Part model, mm, in its own coordinate system. A direction names the side the tool comes from. Give positions to 0.01 mm unless a question says otherwise; leave off trailing zeros. Loops run counter-clockwise (first coordinate to the right, second up) from the corner with the lowest first, then second, coordinate; pieces in that order, holes last. Notation, with made-up numbers: M 5,77 L 36,77 A36 cw 36,114 Z; hole C -6.75,-33.5 d1. An arc over 180 degrees is marked long. Answer in a Markdown table with one row per item.
from build123d import *

# Parameters (mm, degrees)
SKETCH_1_W             = 100
SKETCH_1_H             = 95
EXTRUDE_1_DEPTH        = 25
SKETCH_2_R             = 31
CUT_EXTRUDE_1_DEPTH    = 22
SKETCH_3_R             = 27
CUT_EXTRUDE_2_DEPTH    = 73.389571072
CUT_EXTRUDE_START      = 16
SKETCH_4_R             = 32.5
CUT_EXTRUDE_3_DEPTH    = 2.1
HOLE_WIZARD_M8_1_D     = 6.8
HOLE_WIZARD_M8_1_DEPTH = 15.75
HOLE_WIZARD_M8_1_TIP   = 2.042926105
HOLE_WIZARD_M8_2_D     = 6.8
HOLE_WIZARD_M8_2_DEPTH = 15.75
HOLE_WIZARD_M8_2_TIP   = 2.042926105
CHAMFER_1_SIZE         = 10
CHAMFER_2_SIZE         = 1
HOLE_WIZARD_M8_3_D     = 6.8
HOLE_WIZARD_M8_3_DEPTH = 19.75
HOLE_WIZARD_M8_3_TIP   = 2.042926105


with BuildPart() as part:
    # 草图1 → 凸台-拉伸1 (new body)
    with BuildSketch(Plane(origin=(0, 0, 0), x_dir=(0, 0, -1), z_dir=(1, 0, 0))):
        Rectangle(SKETCH_1_W, SKETCH_1_H)
    extrude(amount=EXTRUDE_1_DEPTH)

    # 草图2 → 切除-拉伸1 (cut)
    with BuildSketch(Plane.ZY):
        with Locations((0, 7.5)):
            Circle(SKETCH_2_R)
    extrude(amount=-CUT_EXTRUDE_1_DEPTH, mode=Mode.SUBTRACT)

    # 草图3 → 切除-拉伸2 (cut, through all)
    with BuildSketch(Plane.ZY.offset(-22)):
        with Locations((0, 7.5)):
            Circle(SKETCH_3_R)
    extrude(amount=-CUT_EXTRUDE_2_DEPTH, mode=Mode.SUBTRACT)

    # 草图4 → 切除-拉伸3 (cut)
    with BuildSketch(Plane.ZY.offset(-22).offset(CUT_EXTRUDE_START)):
        with Locations((0, 7.5)):
            Circle(SKETCH_4_R)
    extrude(amount=CUT_EXTRUDE_3_DEPTH, mode=Mode.SUBTRACT)

    # M8 螺纹孔1
    with Locations(Plane.XY.offset(50)):
        with Locations((12.5, 17.5)):
            Hole(HOLE_WIZARD_M8_1_D / 2, depth=HOLE_WIZARD_M8_1_DEPTH)
            with Locations((0, 0, -(HOLE_WIZARD_M8_1_DEPTH + HOLE_WIZARD_M8_1_TIP / 2))):  # 118° drill point
                Cone(0, HOLE_WIZARD_M8_1_D / 2, HOLE_WIZARD_M8_1_TIP, mode=Mode.SUBTRACT)

    # M8 螺纹孔2
    with Locations(Plane(origin=(0, 0, -50), x_dir=(-1, 0, 0), z_dir=(0, 0, -1))):
        with Locations((-12.5, 17.5)):
            Hole(HOLE_WIZARD_M8_2_D / 2, depth=HOLE_WIZARD_M8_2_DEPTH)
            with Locations((0, 0, -(HOLE_WIZARD_M8_2_DEPTH + HOLE_WIZARD_M8_2_TIP / 2))):  # 118° drill point
                Cone(0, HOLE_WIZARD_M8_2_D / 2, HOLE_WIZARD_M8_2_TIP, mode=Mode.SUBTRACT)

    # 倒角1
    chamfer_1_edges = [part.edges().sort_by_distance(p)[0] for p in [
        (12.5, 47.5, 50),
        (12.5, 47.5, -50),
    ]]
    chamfer(chamfer_1_edges, length=CHAMFER_1_SIZE)

    # 倒角2
    chamfer_2_edges = [part.edges().sort_by_distance(p)[0] for p in [
        (12.5, -47.5, -50),
        (12.5, -47.5, 50),
    ]]
    chamfer(chamfer_2_edges, length=CHAMFER_2_SIZE)

    # M8 螺纹孔3
    with Locations(Plane(origin=(0, -47.5, 0), x_dir=(-1, 0, 0), z_dir=(0, -1, 0))):
        with Locations((-12.5, -40), (-12.5, 0), (-12.5, 40)):
            Hole(HOLE_WIZARD_M8_3_D / 2, depth=HOLE_WIZARD_M8_3_DEPTH)
            with Locations((0, 0, -(HOLE_WIZARD_M8_3_DEPTH + HOLE_WIZARD_M8_3_TIP / 2))):  # 118° drill point
                Cone(0, HOLE_WIZARD_M8_3_D / 2, HOLE_WIZARD_M8_3_TIP, mode=Mode.SUBTRACT)


solid = part.part
(1) Drill centre lines: line 1 along Z through (x, y) = (12.5, -33.25); line 2 along Z through (x, y) = (13, -26.5); line 3 along X through (y, z) = (17.5, -43.75). Where is each one in solid material? Low to high.
Recorded:
| item | result |
|---|---|
| line 1 | z = -50 to -43.4, -36.6 to -3.4, 3.4 to 36.6, 43.4 to 50 |
| line 2 | z = -50 to -41.22, -38.78 to -1.22, 1.22 to 38.78, 41.22 to 50 |
| line 3 | x = 0 to 9.1, 15.9 to 25 |
(2) Pull direction Y, two halves, no side cores. Call faces 4 (the face through (12.06, -37.49, 36.63)), 5 (the face through (12.183, 17.998, -32.562)), 6 (the face through (11.955, -26.062, 0.226)): +Y half, -Y half, draft (parallel to the pull), parting line (faces both ways), or undercut.
Recorded:
| item | result |
|---|---|
| face 4 | draft |
| face 5 | undercut |
| face 6 | -Y half |
(3) Which spindle directions (+Z, -Z, +X, -X, +Y, -Y) get a long thin tool onto all of the face, cutting with end or side? Do faces 1 (the face through (1.923, -22.763, -6.72)), 2 (the face through (6, -4, 29)), 3 (the face through (13.24, 14.18, 42.01)). Say none if no direction does.
Recorded:
| item | result |
|---|---|
| face 1 | -X |
| face 2 | none |
| face 3 | +Z |
(4) Saw through at B-B (y = 7.5). Write the cut outline in (x, z), plus the area to 3 significant figures.
Recorded:
| item | result |
|---|---|
| outline | M 0,-50 L 25,-50 L 25,-27 L 22,-27 L 22,-31 L 6,-31 L 6,-32.5 L 3.9,-32.5 L 3.9,-31 L 0,-31 Z; M 0,31 L 3.9,31 L 3.9,32.5 L 6,32.5 L 6,31 L 22,31 L 22,27 L 25,27 L 25,50 L 0,50 Z |
| area | 968 mm^2 |
(5) Pin check, flat tips, straight feed: pin 1 Ø6 at (y, z) = (22.5, -15) entering from +X; pin 2 Ø6 at (x, z) = (12.5, -40) entering from -Y; pin 3 Ø6 at (x, y) = (12.5, 17.5) entering from -Z; pin 4 Ø4 at (y, z) = (1, -28) entering from -X. Stop position of each tip, or through.
Recorded:
| item | result |
|---|---|
| pin 1 | passes through |
| pin 2 | stops at y = -27.51 |
| pin 3 | stops at z = -34.01 |
| pin 4 | stops at x = 22 |
(6) Saw through at C-C (y = -31). Write the cut outline in (x, z).
Recorded:
| item | result |
|---|---|
| outline | M 0,-50 L 25,-50 L 25,50 L 0,50 Z; hole C 12.5,-40 d6.8; hole C 12.5,0 d6.8; hole C 12.5,40 d6.8 |
(7) Saw through at A-A (z = 15). Write the cut outline in (x, y), plus the area to 3 significant figures.
Recorded:
| item | result |
|---|---|
| outline | M 0,-47.5 L 25,-47.5 L 25,-14.95 L 22,-14.95 L 22,-19.63 L 6,-19.63 L 6,-21.33 L 3.9,-21.33 L 3.9,-19.63 L 0,-19.63 Z; M 0,34.63 L 3.9,34.63 L 3.9,36.33 L 6,36.33 L 6,34.63 L 22,34.63 L 22,29.95 L 25,29.95 L 25,47.5 L 0,47.5 Z |
| area | 1,040 mm^2 |
(8) Saw through at D-D (z = -29). Write the cut outline in (x, y), plus the area to 3 significant figures.
Recorded:
| item | result |
|---|---|
| outline | M 0,-47.5 L 25,-47.5 L 25,47.5 L 0,47.5 L 0,18.45 L 3.9,18.45 L 3.9,22.17 L 6,22.17 L 6,18.45 L 22,18.45 L 22,-3.45 L 6,-3.45 L 6,-7.17 L 3.9,-7.17 L 3.9,-3.45 L 0,-3.45 Z |
| area | 1,880 mm^2 |
